Can you work these out from the model? Positions are in its coordinate system, mm. Face numbers are marked on the shaded views. A direction names the side the tool comes from. Give positions to 0.01 mm unless a question says otherwise; leave off trailing zeros. Order: outer loops, then holes, each group sorted by start corner. A loop starts at its lowest first (then second) coordinate and runs counter-clockwise, first axis right, second up.
Item 1: I want a section at C-C, the plane y = 20. Write out the boundary of the cut face in (x, z), then the cut area to 3 significant figures.
Item 2: Which directions (+Z, -Z, +X, -X, +Y, -Y) give clear straight access to the entire face, cutting with the end or side of a thin tool? Please do the marked faces 1, 2, 3, 4 and 5.
Item 3: I want a section at D-D, the plane y = 1.5. Write out the boundary of the cut face in (x, z).
Item 4: I'm going to push flat-ended pins straight in: pin 1 Ø12 at (y, z) = (17, 20.5) entering from +X; pin 2 Ø1.5 at (y, z) = (27, 14) entering from +X; pin 3 Ø3.5 at (y, z) = (16, 21) entering from -X. Where does each tip first touch, or does it pass through?
Item 5: If we mould it in two halves opening along Z, with no side actions, what happens to the marked faces 6, 7 and 8? For each: +Z half, -Z half, draft (parallel to the pull), parting line (faces both ways), or undercut.
Item 6: I want a section at A-A, the plane x = -32. Write out the boundary of the cut face in (y, z), then the cut area to 3 significant figures.
Item 7: I want a section at B-B, the plane z = -13. Write out the boundary of the cut face in (x, y), then the cut area to 3 significant figures.
Item 8: If I drill on line 1 along Z through (x, y) = (-16, 13.5); line 2 along X through (y, z) = (2, -13); line 3 along Y through (x, z) = (-32, 20.75), over which ranges is the centre line in solid material (lowest first)?
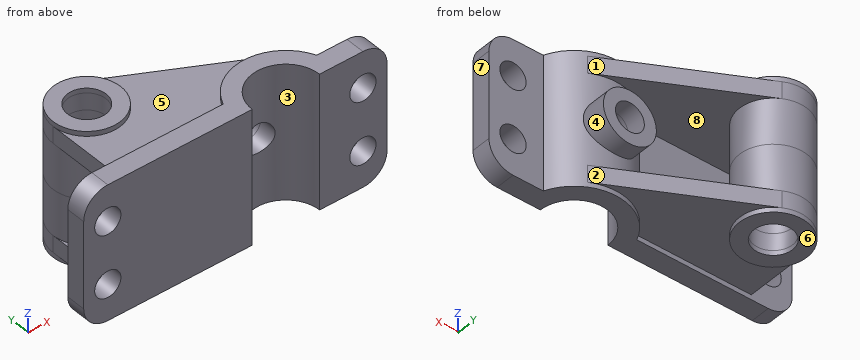
```python
from build123d import *
from build123d.topology import SkipClean

# Parameters (mm, degrees)
BASE_PLATE_SKETCH_R      = 5.452465884
BASE_PLATE_DEPTH         = 4
PIVOT_HOUSING_SKETCH_R   = 14
PIVOT_HOUSING_SKETCH_R_2 = 8
PIVOT_HOUSING_DEPTH      = 28
SADDLE_CUT_SKETCH_R      = 14
SADDLE_CUT_28_DEPTH      = 28
SIDE_WEB_SKETCH_R        = 8
SIDE_WEB_DEPTH           = 7
TOP_BOSS_22_REACH        = 76.411
TOP_BOSS_22_END_RADIUS   = 21
TOP_BOSS_SKETCH_R        = 11
TOP_BOSS_SKETCH_R_2      = 6
TOP_BOSS_HOLE_CUT_REACH  = 76.411
TOP_BOSS_HOLE_SKETCH_R   = 6


with BuildPart() as part:
    # Base Plate Sketch → Base Plate (new, symmetric)
    with BuildSketch(Plane(origin=(0, 0, 0), x_dir=(1, 0, 0), z_dir=(0, 1, 0))):
        with BuildLine():
            Line((-53, 28), (53, 28))
            ThreePointArc((53, 28), (60.071067812, 25.071067812), (63, 18))
            Line((63, 18), (63, -18))
            ThreePointArc((63, -18), (60.071067812, -25.071067812), (53, -28))
            Line((53, -28), (-53, -28))
            ThreePointArc((-53, -28), (-60.071067812, -25.071067812), (-63, -18))
            Line((-63, -18), (-63, 18))
            ThreePointArc((-63, 18), (-60.071067812, 25.071067812), (-53, 28))
        make_face()
        with Locations(Location((-53, 13, 0), (0, 0, 270))):
            Circle(BASE_PLATE_SKETCH_R, mode=Mode.SUBTRACT)
        with Locations(Location((-53, -13, 0), (0, 0, 90))):
            Circle(BASE_PLATE_SKETCH_R, mode=Mode.SUBTRACT)
        with Locations(Location((53, -13, 0), (0, 0, 270))):
            Circle(BASE_PLATE_SKETCH_R, mode=Mode.SUBTRACT)
        with Locations(Location((53, 13, 0), (0, 0, 90))):
            Circle(BASE_PLATE_SKETCH_R, mode=Mode.SUBTRACT)
    extrude(amount=BASE_PLATE_DEPTH, both=True)

    # Pivot Housing Sketch → Pivot Housing (add, symmetric)
    # profile 1 of 2: a face of its own
    with BuildSketch(Plane.XY):
        with Locations((-32, 31.911479001)):
            Circle(PIVOT_HOUSING_SKETCH_R)
        with Locations((-32, 31.911479001)):
            Circle(PIVOT_HOUSING_SKETCH_R_2, mode=Mode.SUBTRACT)
    # profile 2 of 2: a face of its own
    with BuildSketch(Plane.XY):
        with BuildLine():
            Line((0, -4), (7, -4))
            ThreePointArc((7, -4), (21, 10), (35, -4))
            Line((35, -4), (42, -4))
            ThreePointArc((42, -4), (21, 17), (0, -4))
        make_face()
    extrude(amount=PIVOT_HOUSING_DEPTH, both=True)


with BuildPart() as pivot_housing_piece_1:
    # of the separate pieces the step leaves, piece 1, a body of its own (pivot_housing_pieces)
    add(part.part.solids().sort_by_distance((-53, -4, -28))[0])

    # Saddle Cut Sketch → Saddle Cut Ø28 (cut, symmetric)
    with SkipClean():  # the faces are left unmerged after this step: merging them gives an invalid solid
        with BuildSketch(Plane.XY):
            with Locations((21, -4)):
                Circle(SADDLE_CUT_SKETCH_R)
        extrude(amount=SADDLE_CUT_28_DEPTH, both=True, mode=Mode.SUBTRACT)



with BuildPart() as pivot_housing_piece_2:
    # of the separate pieces the step leaves, piece 2, a body of its own (pivot_housing_pieces)
    add(part.part.solids().sort_by_distance((-18, 31.911479001, -28))[0])


with BuildPart() as pivot_housing_piece_1_1:
    with SkipClean():  # the faces are left unmerged after this step: merging them gives an invalid solid
        add(pivot_housing_piece_1.part)

        add(pivot_housing_piece_2.part)  # Side Web merges Pivot Housing piece 2
        # Side Web Sketch → Side Web (add)
        with BuildSketch(Plane.XY.offset(26)):
            with BuildLine():
                Line((-46, 4), (1.583512161, 4))
                ThreePointArc((1.583512161, 4), (13.858235624, 15.748296169), (30.808163701, 14.568788997))
                Line((30.808163701, 14.568788997), (-25.4612242, 44.290671665))
                ThreePointArc((-25.4612242, 44.290671665), (-39.22693361, 43.901951494), (-46, 31.911479001))
                Line((-46, 31.911479001), (-46, 4))
            make_face()
            with Locations((-32, 31.911479001)):
                Circle(SIDE_WEB_SKETCH_R, mode=Mode.SUBTRACT)
        side_web = extrude(amount=-SIDE_WEB_DEPTH)

    # Side Web Mirror: Side Web across plane
    with SkipClean():  # the faces are left unmerged after this step: merging them gives an invalid solid
        add(side_web.mirror(Plane.XY))

    # Top Boss Ø22: up to this cylinder (the profile starts outside it)
    with SkipClean():  # the faces are left unmerged after this step: merging them gives an invalid solid
        top_boss_22_end = Plane(origin=(21, -4, -10.688873), z_dir=(0, 0, -1)) * Cylinder(TOP_BOSS_22_END_RADIUS, 195.822, mode=Mode.PRIVATE)
        # Top Boss Sketch → Top Boss Ø22 (add, up to the surface)
        with BuildSketch(Plane(origin=(0, 24, 0), x_dir=(1, 0, 0), z_dir=(0, 1, 0)), mode=Mode.PRIVATE) as top_boss_22_sk1:
            with Locations(Location((21, 0, 0), (0, 0, 270))):
                Circle(TOP_BOSS_SKETCH_R)
            with Locations(Location((21, 0, 0), (0, 0, 270))):
                Circle(TOP_BOSS_SKETCH_R_2, mode=Mode.SUBTRACT)
        top_boss_22_tool1 = extrude(top_boss_22_sk1.sketch, amount=-TOP_BOSS_22_REACH, mode=Mode.PRIVATE) - top_boss_22_end
        add(top_boss_22_tool1.solids().sort_by_distance((21, 24, -10.688873))[0])

    # Top Boss Hole Sketch → Top Boss Hole Cut (cut, up to next)
    with BuildSketch(Plane(origin=(0, 24, 0), x_dir=(1, 0, 0), z_dir=(0, 1, 0)), mode=Mode.PRIVATE) as top_boss_hole_cut_sk1:
        with Locations(Location((21, 0, 0), (0, 0, 270))):
            Circle(TOP_BOSS_HOLE_SKETCH_R)
    top_boss_hole_cut_tool1 = extrude(top_boss_hole_cut_sk1.sketch, amount=-TOP_BOSS_HOLE_CUT_REACH, mode=Mode.PRIVATE) & pivot_housing_piece_1_1.part
    add(top_boss_hole_cut_tool1.solids().sort_by_distance((21, 24, 0))[0], mode=Mode.SUBTRACT)


solid = pivot_housing_piece_1_1.part
```
Results list:
1. outline: (-46, -26) - (-39.36, -26) - (-39.36, -28) - (-24.64, -28) - (-24.64, -26) - (20.53, -26) - (20.53, -19) - (-24.64, -19) - (-24.64, 19) - (20.53, 19) - (20.53, 26) - (-24.64, 26) - (-24.64, 28) - (-39.36, 28) - (-39.36, 26) - (-46, 26) - (-46, 19) - (-39.36, 19) - (-39.36, -19) - (-46, -19) - close; circle Ø22 at (21, 0); hole circle Ø12 at (21, 0)
1. area: 1,820 mm2
2. face 1: +Z, +X, +Y
2. face 2: -Z, +X, +Y
2. face 3: +Z, -Z, -Y
2. face 4: +Y
2. face 5: +Z
3. outline: (-63, -18) arc R10 ccw to (-53, -28) - (8.13, -28) - (8.13, 28) - (-53, 28) arc R10 ccw to (-63, 18) - close; (33.87, -28) - (53, -28) arc R10 ccw to (63, -18) - (63, 18) arc R10 ccw to (53, 28) - (33.87, 28) - close; hole circle Ø10.9 at (-53, -13); hole circle Ø10.9 at (-53, 13); hole circle Ø10.9 at (53, -13); hole circle Ø10.9 at (53, 13)
4. pin 1: stops at x = 35.7
4. pin 2: stops at x = -18.63
4. pin 3: stops at x = -46
5. face 6: -Z half
5. face 7: draft
5. face 8: undercut
6. outline: (-4, -28) - (4, -28) - (4, -26) - (17.91, -26) - (17.91, -28) - (23.91, -28) - (23.91, 28) - (17.91, 28) - (17.91, 26) - (4, 26) - (4, 28) - (-4, 28) - close; (39.91, -28) - (45.91, -28) - (45.91, 28) - (39.91, 28) - close; hole (4, -19) - (17.91, -19) - (17.91, 19) - (4, 19) - close
6. area: 1,310 mm2
7. outline: (-63, -4) - (-58.45, -4) - (-58.45, 4) - (-63, 4) - close; (-47.55, -4) - (7, -4) arc R14 cw to (35, -4) - (47.55, -4) - (47.55, 4) - (40.42, 4) arc R21 ccw to (1.58, 4) - (-47.55, 4) - close; circle Ø28 at (-32, 31.91); (58.45, -4) - (63, -4) - (63, 4) - (58.45, 4) - close; hole circle Ø16 at (-32, 31.91)
7. area: 1,310 mm2
8. line 1: z = -26 to -19, 19 to 26
8. line 2: x = -63 to -58.45, -47.55 to 8.35, 33.65 to 47.55, 58.45 to 63
8. line 3: y = -4 to 23.91, 39.91 to 45.91
